from build123d import *

# Parameters (mm, degrees)
SKETCH_1_W          = 85
SKETCH_1_H          = 85
SKETCH_1_R          = 36
EXTRUDE_1_DEPTH     = 4
HOLE_WIZARD_M6_1_D  = 5
SKETCH_4_W          = 85
SKETCH_4_H          = 8
EXTRUDE_2_DEPTH     = 30
CUT_EXTRUDE_1_DEPTH = 95.293425009


with BuildPart() as part:
    # 草图1 → 凸台-拉伸1 (new, symmetric)
    with BuildSketch(Plane.XY):
        Rectangle(SKETCH_1_W, SKETCH_1_H)
        with Locations((0, 2.5)):
            Circle(SKETCH_1_R, mode=Mode.SUBTRACT)
    extrude(amount=EXTRUDE_1_DEPTH, both=True)

    # M6 螺纹孔1 (through all)
    with Locations(Plane(origin=(-31.819805153, 34.319805153, 4), x_dir=(1, 0, 0), z_dir=(0, 0, 1))):
        with Locations((0, 0), (63.639610306, -63.639610306), (0, -63.639610306), (63.639610306, 0)):
            Hole(HOLE_WIZARD_M6_1_D / 2)

    # 草图4 → 凸台-拉伸2 (add)
    with BuildSketch(Plane.XY.offset(4)):
        with Locations((0, -38.5)):
            Rectangle(SKETCH_4_W, SKETCH_4_H)
    extrude(amount=EXTRUDE_2_DEPTH)

    # 草图5 → 切除-拉伸1 (cut, through all)
    with BuildSketch(Plane(origin=(0, -34.5, 0), x_dir=(1, 0, 0), z_dir=(0, 1, 0))):
        with BuildLine():
            Line((-32.5, -20.75), (-17.5, -20.75))
            ThreePointArc((-17.5, -20.75), (-14.25, -24), (-17.5, -27.25))
            Line((-17.5, -27.25), (-32.5, -27.25))
            ThreePointArc((-32.5, -27.25), (-35.75, -24), (-32.5, -20.75))
        make_face()
        with BuildLine():
            Line((17.5, -20.75), (32.5, -20.75))
            ThreePointArc((32.5, -20.75), (35.75, -24), (32.5, -27.25))
            Line((32.5, -27.25), (17.5, -27.25))
            ThreePointArc((17.5, -27.25), (14.25, -24), (17.5, -20.75))
        make_face()
    extrude(amount=-CUT_EXTRUDE_1_DEPTH, mode=Mode.SUBTRACT)


solid = part.part
Work out the finished part from the listing and answer in its coordinate system (mm). A direction names the side the tool comes from. Give positions to 0.01 mm unless a question says otherwise; leave off trailing zeros. Loops run counter-clockwise (first coordinate to the right, second up) from the corner with the lowest first, then second, coordinate; pieces in that order, holes last. Notation, with made-up numbers: (3.25, 64.5) -> (61.25, 64.5) arc R17 cw to (61.25, 76.5) -> close; hole circle Ø6 at (-27.5, 29.5). An arc over 180 degrees is marked (long way). Use a Markdown table: item, result. Add a question column.
1) Which of the six approach directions +Z, -Z, +X, -X, +Y, -Y give full straight-line access (tool end or side, diameter ignored) to faces 1 (the cylindrical face through (-29.322, 34.43, -0.056)), 2 (the flat face through (25, -38, 20.75))?
2) The part is cut by section D-D, the plane x = -16. Determine the outline of the cut face in (y, z), plus the area to 3 significant figures.
3) Consider line 1 along Y through (x, z) = (0, -1); line 2 along Z through (x, y) = (-32.5, -17); line 3 along Y through (x, z) = (-36, 26). Determine where each line is inside the solid, lowest interval first.
4) The part is cut by section B-B, the plane x = 0. Determine the outline of the cut face in (y, z), plus the area to 3 significant figures.
5) The part is cut by section A-A, the plane z = 24. Determine the outline of the cut face in (x, y).
6) The part is cut by section C-C, the plane y = 2.5. Determine the outline of the cut face in (x, z), plus the area to 3 significant figures.
7) Each of these flat-tipped pins is pushed along its axis until it touches: P1, Ø2, axis at x = -6.5, z = 18, coming from the +Y side; P2, Ø6, axis at x = 31.82, y = -29.32, coming from the +Z side. Where does it stop, or does it pass through?
8) For a pull along Z with two mould halves and no side action, classify faces 3 (the cylindrical face through (14.25, -38.44, 24.07)), 4 (the flat face through (-1, -42.5, 15)), 5 (the flat face through (-1, 39, 4)) as +Z half, -Z half, draft (parallel to the pull), parting line (faces both ways), or undercut.
Reported:
| question | item | result |
|---|---|---|
| 1 | face 1 | +Z, -Z |
| 1 | face 2 | +Y, -Y |
| 2 | outline | (-42.5, -4) -> (-29.75, -4) -> (-29.75, 4) -> (-34.5, 4) -> (-34.5, 21.12) -> (-42.5, 21.12) -> close; (-42.5, 26.88) -> (-34.5, 26.88) -> (-34.5, 34) -> (-42.5, 34) -> close; (34.75, -4) -> (42.5, -4) -> (42.5, 4) -> (34.75, 4) -> close |
| 2 | area | 358 mm^2 |
| 3 | line 1 | y = -42.5 to -33.5, 38.5 to 42.5 |
| 3 | line 2 | z = -4 to 4 |
| 3 | line 3 | y = -42.5 to -34.5 |
| 4 | outline | (-42.5, -4) -> (-33.5, -4) -> (-33.5, 4) -> (-34.5, 4) -> (-34.5, 34) -> (-42.5, 34) -> close; (38.5, -4) -> (42.5, -4) -> (42.5, 4) -> (38.5, 4) -> close |
| 4 | area | 344 mm^2 |
| 5 | outline | (-42.5, -42.5) -> (-35.75, -42.5) -> (-35.75, -34.5) -> (-42.5, -34.5) -> close; (-14.25, -42.5) -> (14.25, -42.5) -> (14.25, -34.5) -> (-14.25, -34.5) -> close; (35.75, -42.5) -> (42.5, -42.5) -> (42.5, -34.5) -> (35.75, -34.5) -> close |
| 6 | outline | (-42.5, -4) -> (-36, -4) -> (-36, 4) -> (-42.5, 4) -> close; (36, -4) -> (42.5, -4) -> (42.5, 4) -> (36, 4) -> close |
| 6 | area | 104 mm^2 |
| 7 | P1 | stops at y = -34.5 |
| 7 | P2 | stops at z = 4 |
| 8 | face 3 | undercut |
| 8 | face 4 | draft |
| 8 | face 5 | +Z half |
